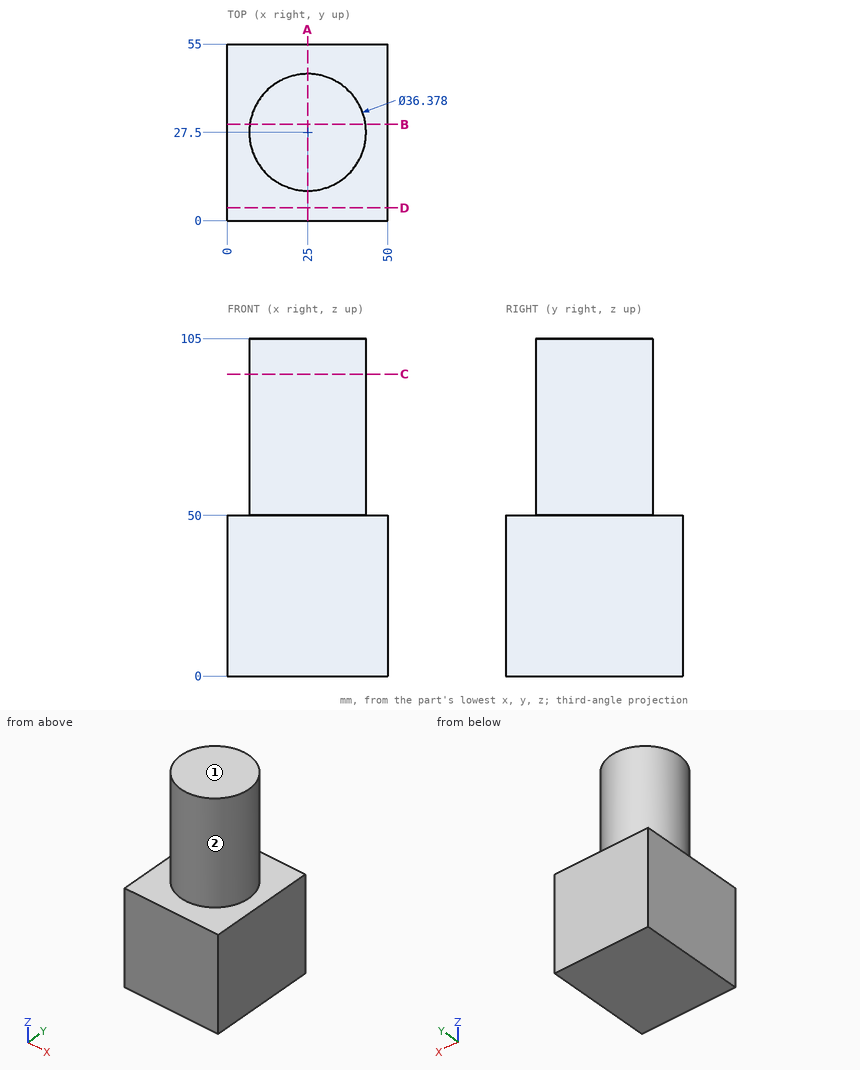
Print and shaded views of the part. All mm, measured from the part's lowest x, y and z. A direction names the side the tool comes from. Round coordinates to 2 decimals unless told otherwise and drop trailing zeros. Order: outer loops, then holes, each group sorted by start corner. A loop starts at its lowest first (then second) coordinate and runs counter-clockwise, first axis right, second up.
Q1. Which spindle directions (+Z, -Z, +X, -X, +Y, -Y) get a long thin tool onto all of the face, cutting with end or side? Do the marked faces 1 and 2. Say none if no direction does.
Q2. Drop flat-ended pins along their axis: pin 1 (1 mm diameter, centred on x = 20, z = 92, fed in from -Y); pin 2 (10 mm diameter, centred on x = 22, z = 69.5, fed in from +Y); pin 3 (4 mm diameter, centred on y = 20, z = 63.5, fed in from +X). Give the stop position or say it passes through.
Q3. Slice it at C-C (z = 94). Write the cut outline in (x, y), and give its area (3 significant figures).
Q4. Slice it at A-A (x = 25). Write the cut outline in (y, z), and give its area (3 significant figures).
Q5. Slice it at D-D (y = 4). Write the cut outline in (x, z), and give its area (3 significant figures).
Q6. Wall check: L1, parallel to Z at x = 37, y = 10; L2, parallel to Y at x = 18, z = 76.5; L3, parallel to X at y = 14.5, z = 59. Give the ranges that are in metal, low to high.
Q7. Slice it at B-B (y = 30). Write the cut outline in (x, z).
Results below:
1. face 1: +Z, +X, -X, +Y, -Y
1. face 2: +Z
2. pin 1: stops at y = 9.88
2. pin 2: stops at y = 45.69
2. pin 3: stops at x = 42.34
3. outline: circle Ø36.38 at (25, 27.5)
3. area: 1,040 mm2
4. outline: (0, 0) - (55, 0) - (55, 50) - (45.69, 50) - (45.69, 105) - (9.31, 105) - (9.31, 50) - (0, 50) - close
4. area: 4,750 mm2
5. outline: (0, 0) - (50, 0) - (50, 50) - (0, 50) - close
5. area: 2,500 mm2
6. L1: z = 0 to 50
6. L2: y = 10.71 to 44.29
6. L3: x = 12.28 to 37.72
7. outline: (0, 0) - (50, 0) - (50, 50) - (43.02, 50) - (43.02, 105) - (6.98, 105) - (6.98, 50) - (0, 50) - close
